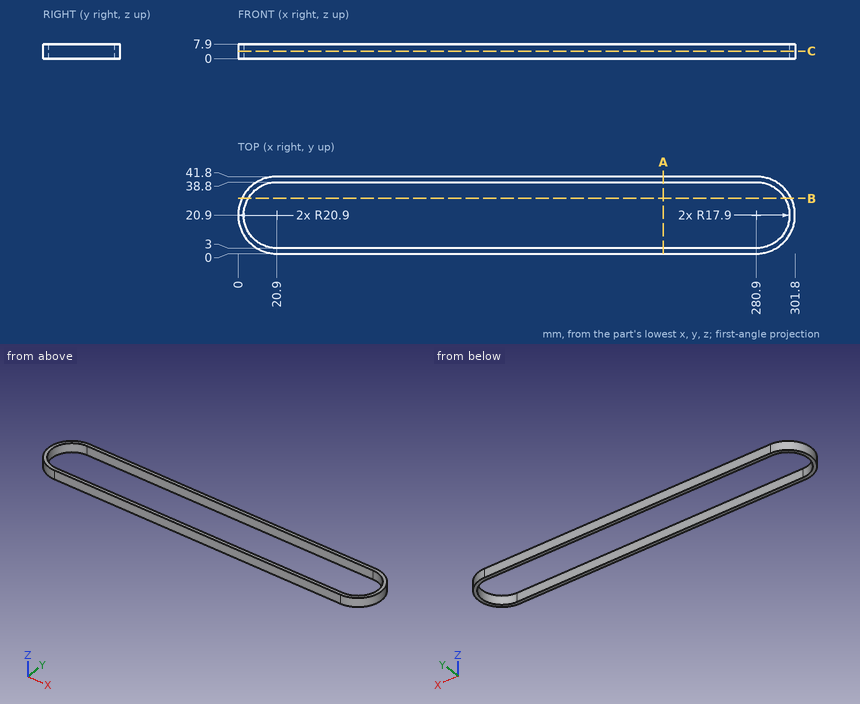
Here's the drawing with two shaded views (mm, measured from the low corner). I have some questions. Give positions to 0.01 mm unless a question says otherwise; leave off trailing zeros. Loops run counter-clockwise (first coordinate to the right, second up) from the corner with the lowest first, then second, coordinate; pieces in that order, holes last. Notation, with made-up numbers: (5, 86) - (26, 86) arc R27 ccw to (26, 105) - close; hole circle Ø1 at (32, -38.5). An arc over 180 degrees is marked (long way). Return JSON: item names as keys, results as strings.
1. I want a section at A-A on x = 230.5. Please give me the cut outline in (y, z).
Output values:
{"outline": "(0, 0) - (3, 0) - (3, 7.9) - (0, 7.9) - close; (38.8, 0) - (41.8, 0) - (41.8, 7.9) - (38.8, 7.9) - close"}
2. I want a section at C-C on z = 4. Please give me the cut outline in (x, y), and give its area (3 significant figures).
Output values:
{"outline": "(20.9, 0) - (280.9, 0) arc R20.9 ccw to (280.9, 41.8) - (20.9, 41.8) arc R20.9 ccw to start; hole (20.9, 3) - (280.9, 3) arc R17.9 ccw to (280.9, 38.8) - (20.9, 38.8) arc R17.9 ccw to start", "area": "1,930 mm²"}
3. If I drill on line 1 (Y direction, x = 37.5, z = 3.25); line 2 (X direction, y = 9.5, z = 7.5); line 3 (X direction, y = 24, z = 5), over which ranges is the centre line in solid material (lowest first)?
Output values:
{"line 1": "y = 0 to 3, 38.8 to 41.8", "line 2": "x = 3.38 to 7.1, 294.7 to 298.42", "line 3": "x = 0.23 to 3.27, 298.53 to 301.57"}
4. I want a section at B-B on y = 30. Please give me the cut outline in (x, z).
Output values:
{"outline": "(2.09, 0) - (5.49, 0) - (5.49, 7.9) - (2.09, 7.9) - close; (296.31, 0) - (299.71, 0) - (299.71, 7.9) - (296.31, 7.9) - close"}
